from build123d import *

# Parameters (mm, degrees)
SQUARE_DRIVE_SKETCH_OUTSIDE_W = 29.184
SQUARE_DRIVE_SKETCH_OUTSIDE_H = 29.184
SQUARE_DRIVE_5X5_CUT_DEPTH    = 6


with BuildPart() as part:
    # Spindle Profile Sketch → Spindle Body Revolve (revolve)
    with BuildSketch(Plane.XY, mode=Mode.PRIVATE) as spindle_body_revolve_sk:
        Polygon((0, 0), (0, 2.5), (-6, 2.5), (-6, 3), (-44, 3), (-44, 4), (-56, 4), (-56, 3), (-66, 3), (-68, 6), (-70.535898385, 6), (-74, 0), align=None)
    revolve(spindle_body_revolve_sk.sketch.rotate(Axis((0, 0, 0), (-1, 0, 0)), 90), axis=Axis((0, 0, 0), (-1, 0, 0)))

    # Square Drive Sketch outside → Square Drive 5x5 Cut (cut)
    with BuildSketch(Plane(origin=(0, 0, 0), x_dir=(0, 0, -1), z_dir=(1, 0, 0))):
        Rectangle(SQUARE_DRIVE_SKETCH_OUTSIDE_W, SQUARE_DRIVE_SKETCH_OUTSIDE_H)
        Polygon((-0.5, 2.5), (-2.5, 0.5), (-2.5, -0.5), (-0.5, -2.5), (0.5, -2.5), (2.5, -0.5), (2.5, 0.5), (0.5, 2.5), align=None, mode=Mode.SUBTRACT)
    extrude(amount=-SQUARE_DRIVE_5X5_CUT_DEPTH, mode=Mode.SUBTRACT)


solid = part.part
Here's how the part is built. I have some questions about the finished solid (model axes, mm). A direction names the side the tool comes from. Coordinates: 2 decimals unless noted, no trailing zeros. Order: outer loops, then holes, each group sorted by start corner. A loop starts at its lowest first (then second) coordinate and runs counter-clockwise, first axis right, second up.
Item 1: For P1, Ø6.5, axis at y = 1.5, z = 0.5, coming from the +X side; P2, Ø3, axis at x = -41.5, y = -5, coming from the -Z side; P3, Ø1.5, axis at y = -2.5, z = -3, coming from the -X side; P4, Ø6, axis at x = -45, y = 2.5, coming from the +Z side, each with a flat end and sliding along its axis, tell me the tip position at first contact or that it passes through.
Result sheet:
P1: stops at x = 0
P2: passes through
P3: stops at x = -72.18
P4: stops at z = 4
Item 2: For faces 1 (the face through (-3, -1, 2)), 2 (the face through (-3, 2, 1)), 3 (the face through (-56, -3, -1)), 4 (the face through (-44, -3, 1)), which set-ups out of +Z, -Z, +X, -X, +Y, -Y let a thin tool reach every point of the face, with its end or its side?
Result sheet:
face 1: +Z, +X, -Y
face 2: +Z, +X, +Y
face 3: none
face 4: +X
Item 3: If we mould it in two halves opening along X, with no side actions, what happens to faces 5 (the face through (-6, 2, 2)), 6 (the face through (-73.447, 0.85, -0.442)), 7 (the face through (-3, 1, -2)), 8 (the face through (-61.07, -0.9, -2.86))? For each: +X half, -X half, draft (parallel to the pull), parting line (faces both ways), or undercut.
Result sheet:
face 5: +X half
face 6: -X half
face 7: draft
face 8: undercut
Item 4: I need wall thicknesses on line 1 (X direction, y = -3.25, z = 1.5); line 2 (Y direction, x = -30, z = 0); line 3 (X direction, y = -0.5, z = -3.5). Which ranges of each line are inside material? Lowest first, please.
Result sheet:
line 1: x = -71.93 to -66.39, -56 to -44
line 2: y = -3 to 3
line 3: x = -71.96 to -66.36, -56 to -44
Item 5: If we section it at A-A on x = -25.5: List the corners of the cut face in (y, z) for me.
Result sheet:
outline: circle Ø6 at (0, 0)
